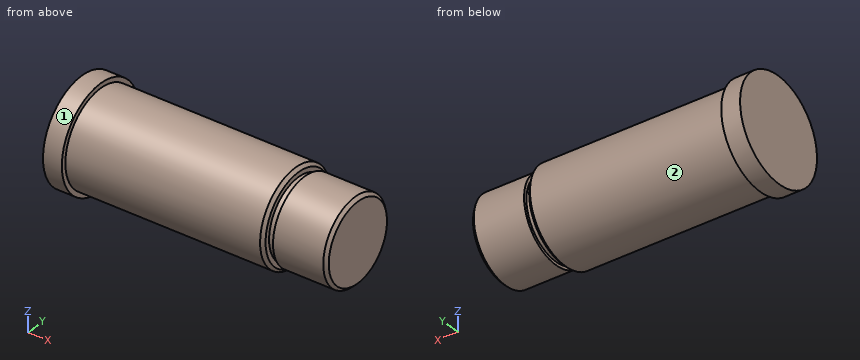
from build123d import *

# Parameters (mm, degrees)
CHAMFER_1_SIZE = 1


with BuildPart() as part:
    # 草图1 → 旋转1 (revolve)
    with BuildSketch(Plane.XY, mode=Mode.PRIVATE) as revolve_1_sk:
        Polygon((0, 0), (0, 16.5), (6, 16.5), (6, 15), (69, 15), (69, 12.5), (71, 12.5), (71, 13.5), (88, 13.5), (88, 0), align=None)
    revolve(revolve_1_sk.sketch.rotate(Axis((0, 0, 0), (1, 0, 0)), 90), axis=Axis((0, 0, 0), (1, 0, 0)))

    # 倒角1
    chamfer_1_edges = [part.edges().sort_by_distance(p)[0] for p in [
        (69, 0, -15),
        (88, 0, -13.5),
    ]]
    chamfer(chamfer_1_edges, length=CHAMFER_1_SIZE)


solid = part.part
The model under review builds one solid part; all positions refer to its coordinate system, in mm. Face numbers are marked on the shaded views. A direction names the side the tool comes from. Round coordinates to 2 decimals unless told otherwise and drop trailing zeros. Write each loop counter-clockwise with the first axis right and the second up, starting at its lowest first coordinate (ties: lowest second). Pieces come first, ordered by that corner, then holes. Notation, with made-up numbers: (42, 9.25) - (61, 9.25) arc R20 cw to (61, 40.25) - close; hole circle Ø3 at (31.5, 34). An arc over 180 degrees is marked (long way). One line per item, written item: value. Start each with the question number.
1. Clearance check with flat-ended pins moving along their axes: P1, Ø4, axis at x = 51.5, y = 7.5, coming from the -Z side; P2, Ø5, axis at x = 61.5, z = 3.5, coming from the +Y side; P3, Ø5, axis at x = 44.5, z = 8.5, coming from the +Y side. State where each tip first meets the part, or that it passes through.
2. Consider section C-C on x = 45. Write out the cut boundary in (y, z).
3. To check wall thickness, follow L1, parallel to X at y = 10.5, z = 7; L2, parallel to X at y = -13, z = 2.5; L3, parallel to X at y = -13, z = -8.5. State the ranges of each line that lie inside material, in increasing order. Write a range as from..to.
4. Consider section A-A on z = 0. Write out the cut boundary in (x, y), and give its area (4 significant figures).
5. Machinability: for the marked faces 1 and 2, which of the approach directions +Z, -Z, +X, -X, +Y, -Y give a long, thin tool a straight path to every point of the face, cutting with its end or side? Answer none if there is none.
Checks:
1. P1: stops at z = -13.96
1. P2: stops at y = 14.97
1. P3: stops at y = 13.75
2. outline: circle Ø30 at (0, 0)
3. L1: x = 0..69, 71..87.88
3. L2: x = 0..69, 71..87.26
3. L3: x = 0..6
4. outline: (0, -16.5) - (6, -16.5) - (6, -15) - (68, -15) - (69, -14) - (69, -12.5) - (71, -12.5) - (71, -13.5) - (87, -13.5) - (88, -12.5) - (88, 12.5) - (87, 13.5) - (71, 13.5) - (71, 12.5) - (69, 12.5) - (69, 14) - (68, 15) - (6, 15) - (6, 16.5) - (0, 16.5) - close
4. area: 2,595 mm^2
5. face 1: +X, -X
5. face 2: +X
